Work out the finished part from the listing and answer in its coordinate system (mm). A direction names the side the tool comes from. Coordinates: 2 decimals unless noted, no trailing zeros. Write each loop counter-clockwise with the first axis right and the second up, starting at its lowest first coordinate (ties: lowest second). Pieces come first, ordered by that corner, then holes. Notation, with made-up numbers: (32, -14) - (56, -14) arc R26 cw to (56, 11) - close; hole circle Ø2 at (-3.75, 85). An arc over 180 degrees is marked (long way). Use a Markdown table: item, result. Add a question column.
(1) The part is cut by section A-A, the plane y = 0. Give the vertices of the cut face in (x, z), then the cut area to 3 significant figures.
(2) Find the intervals of material crossed by line 1 (Y direction, x = 0, z = 1); line 2 (Y direction, x = 0, z = -16.5); line 3 (X direction, y = -7.5, z = 7.5), in increasing order. Write a range as from..to.
(3) The part is cut by section D-D, the plane z = -16.5. Give the vertices of the cut face in (x, y).
(4) For a pull along X with two mould halves and no side action, classify faces 1 (the face through (-4.336, -19.524, 0.28)), 2 (the face through (0, 15, -20.5)), 3 (the face through (6.2, -9.3, 13.5)), 4 (the face through (12.932, -5.362, 16.796)) as released by +X, released by -X, zero draft, split by the parting line, or undercut.
(5) A tool of negligible diameter and unlimited length cuts with its end or side. For faces 5 (the face through (12.932, -5.362, -16.796)), 6 (the face through (-2.38, -10.74, -0.19)), from which of +Z, -Z, +X, -X, +Y, -Y can it reach the whole face along a straight path? Write none if from no direction.
(6) Given pin 1 Ø10 at (y, z) = (-8, -13) entering from +X; pin 2 Ø10 at (x, z) = (12.5, -3.5) entering from +Y; pin 3 Ø3 at (x, z) = (2, 11) entering from -Y, each flat-ended and moving along its own axis, determine where each tip first touches the part or whether it passes through.
(7) The part is cut by section C-C, the plane z = -1. Give the vertices of the cut face in (x, y), then the cut area to 3 significant figures.
from build123d import *

# Parameters (mm, degrees)
SKETCH_2_R          = 20
SKETCH_2_R_2        = 11
EXTRUDE_1_DEPTH     = 20.5
SKETCH_3_R          = 14
CUT_EXTRUDE_1_DEPTH = 7
CHAMFER_3_SIZE      = 0.5


with BuildPart() as part:
    # 草图2 → 凸台-拉伸1 (new, symmetric)
    with BuildSketch(Plane.XY):
        Circle(SKETCH_2_R)
        Circle(SKETCH_2_R_2, mode=Mode.SUBTRACT)
    extrude(amount=EXTRUDE_1_DEPTH, both=True)

    # 草图3 → 切除-拉伸1 (cut)
    with BuildSketch(Plane.XY.offset(20.5)):
        Circle(SKETCH_3_R)
    cut_extrude_1 = extrude(amount=-CUT_EXTRUDE_1_DEPTH, mode=Mode.SUBTRACT)

    # 镜向6: 切除-拉伸1 across plane
    add(cut_extrude_1.mirror(Plane.XY), mode=Mode.SUBTRACT)

    # 倒角3
    chamfer_3_edges = [part.edges().sort_by_distance(p)[0] for p in [
        (-14, 0, 20.5),
        (-14, 0, -20.5),
        (-20, 0, -20.5),
        (-20, 0, 20.5),
    ]]
    chamfer(chamfer_3_edges, length=CHAMFER_3_SIZE)


solid = part.part
Model answer:
| question | item | result |
|---|---|---|
| 1 | outline | (-20, -20) - (-19.5, -20.5) - (-14.5, -20.5) - (-14, -20) - (-14, -13.5) - (-11, -13.5) - (-11, 13.5) - (-14, 13.5) - (-14, 20) - (-14.5, 20.5) - (-19.5, 20.5) - (-20, 20) - close; (11, -13.5) - (14, -13.5) - (14, -20) - (14.5, -20.5) - (19.5, -20.5) - (20, -20) - (20, 20) - (19.5, 20.5) - (14.5, 20.5) - (14, 20) - (14, 13.5) - (11, 13.5) - close |
| 1 | area | 653 mm^2 |
| 2 | line 1 | -20..-11, 11..20 |
| 2 | line 2 | -20..-14, 14..20 |
| 2 | line 3 | -18.54..-8.05, 8.05..18.54 |
| 3 | outline | circle Ø40 at (0, 0); hole circle Ø28 at (0, 0) |
| 4 | face 1 | split by the parting line |
| 4 | face 2 | zero draft |
| 4 | face 3 | undercut |
| 4 | face 4 | undercut |
| 5 | face 5 | -Z |
| 5 | face 6 | +Z, -Z |
| 6 | pin 1 | x = 19.77 |
| 6 | pin 2 | y = 18.54 |
| 6 | pin 3 | y = -19.99 |
| 7 | outline | circle Ø40 at (0, 0); hole circle Ø22 at (0, 0) |
| 7 | area | 877 mm^2 |
